from build123d import *

# Parameters (mm, degrees)
BOSS_EXTRUDE1_DEPTH = 15


with BuildPart() as part:
    # Sketch1 → Boss-Extrude1 (new body)
    with BuildSketch(Plane.XZ):
        Polygon((300, 420), (0, 420), (0, 0), (325, 0), (325, 404), (300, 404), align=None)
    extrude(amount=-BOSS_EXTRUDE1_DEPTH)


solid = part.part
Check sheet for the modelled part. Datum: model origin and axes. Units: mm. A direction names the side the tool comes from. Round coordinates to 2 decimals unless told otherwise and drop trailing zeros.
1. Gauge pin test, flat ends, axial feed: pin 1 Ø6 at (y, z) = (6.5, 278.5) entering from -X; pin 2 Ø7.5 at (y, z) = (6.5, 414) entering from +X. Record the tip position at first contact, or that the pin passes through.
2. Scan line: probe 1 along Z at (x, y) = (309, 12.5). Record every from-to range of solid material in increasing order.
3. Set-up check for faces 1 (the flat face through (313, 7, 404)), 2 (the flat face through (0, 7, 213)): record each of +Z, -Z, +X, -X, +Y, -Y from which the full face is reachable in a straight line by a thin tool's end or side.
Recorded:
1. pin 1: stops at x = 0
1. pin 2: stops at x = 300
2. probe 1: z = 0 to 404
3. face 1: +Z, +X, +Y, -Y
3. face 2: +Z, -Z, -X, +Y, -Y
